```python
from build123d import *

# Parameters (mm, degrees)
SKETCH1_W             = 80
SKETCH1_H             = 105
BOSS_EXTRUDE1_DEPTH   = 3
SKETCH2_R             = 2.6
SKETCH2_R_2           = 15.25
CUT_EXTRUDE1_DEPTH    = 10
M5_TAPPED_HOLE1_D     = 4.2
M5_TAPPED_HOLE1_DEPTH = 12.4
M5_TAPPED_HOLE1_TIP   = 1.2618073
CHAMFER1_SIZE         = 2
SKETCH6_R             = 2.75
CUT_EXTRUDE3_DEPTH    = 133.037873355


with BuildPart() as part:
    # Sketch1 → Boss-Extrude1 (new body)
    with BuildSketch(Plane.XY):
        with Locations((40, 52.5)):
            Rectangle(SKETCH1_W, SKETCH1_H)
    extrude(amount=BOSS_EXTRUDE1_DEPTH)

    # Sketch2 → Cut-Extrude1 (cut)
    with BuildSketch(Plane.XY.offset(3)):
        with Locations((7.5, 97.5)):
            Circle(SKETCH2_R)
        with Locations((72.5, 97.5)):
            Circle(SKETCH2_R)
        with Locations((7.5, 7.5)):
            Circle(SKETCH2_R)
        with Locations((72.5, 7.5)):
            Circle(SKETCH2_R)
        with Locations((40, 65)):
            Circle(SKETCH2_R_2)
    extrude(amount=-CUT_EXTRUDE1_DEPTH, mode=Mode.SUBTRACT)

    # M5 Tapped Hole1
    with Locations(Plane.XY.offset(3)):
        with Locations((11.008621971, 78.991378029), (68.991378029, 78.991378029), (11.008621971, 21.008621971), (68.991378029, 21.008621971)):
            Hole(M5_TAPPED_HOLE1_D / 2, depth=M5_TAPPED_HOLE1_DEPTH)
            with Locations((0, 0, -(M5_TAPPED_HOLE1_DEPTH + M5_TAPPED_HOLE1_TIP / 2))):  # 118° drill point
                Cone(0, M5_TAPPED_HOLE1_D / 2, M5_TAPPED_HOLE1_TIP, mode=Mode.SUBTRACT)

    # Chamfer1
    chamfer1_edges = [part.edges().sort_by_distance(p)[0] for p in [
        (0, 105, 1.5),
        (80, 105, 1.5),
        (80, 0, 1.5),
        (0, 0, 1.5),
    ]]
    chamfer(chamfer1_edges, length=CHAMFER1_SIZE)

    # Sketch6 → Cut-Extrude3 (cut, through all)
    with BuildSketch(Plane(origin=(0, 0, 0), x_dir=(-1, 0, 0), z_dir=(0, 0, -1))):
        with Locations((-68.991378029, 78.991378029)):
            Circle(SKETCH6_R)
        with Locations((-11.008621971, 78.991378029)):
            Circle(SKETCH6_R)
        with Locations((-68.991378029, 21.008621971)):
            Circle(SKETCH6_R)
        with Locations((-11.008621971, 21.008621971)):
            Circle(SKETCH6_R)
    extrude(amount=-CUT_EXTRUDE3_DEPTH, mode=Mode.SUBTRACT)


solid = part.part
```
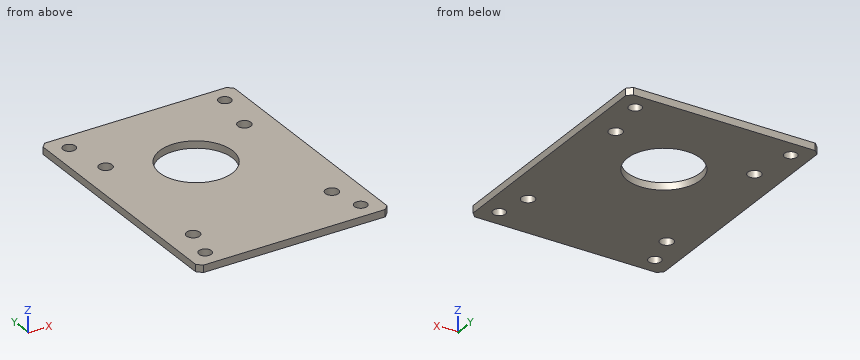
Design review of the part built by this model. Coordinates are the model's own, in mm. Round coordinates to 2 decimals unless told otherwise and drop trailing zeros. Write each loop counter-clockwise with the first axis right and the second up, starting at its lowest first coordinate (ties: lowest second). Pieces come first, ordered by that corner, then holes. Notation, with made-up numbers: (-15.75, -20) -> (21.25, -20) arc R17 cw to (21.25, 6) -> close; hole circle Ø1 at (-3.5, -5). An arc over 180 degrees is marked (long way). Answer in a Markdown table with one row per item.
Q1. To check wall thickness, follow L1, parallel to Y at x = 72.5, z = 1.3; L2, parallel to X at y = 19, z = 2.9; L3, parallel to Y at x = 74.5, z = 1.9. State the ranges of each line that lie inside material, in increasing order. Write a range as [from, to].
The answers:
| item | result |
|---|---|
| L1 | [0, 4.9], [10.1, 94.9], [100.1, 105] |
| L2 | [0, 9.13], [12.89, 67.11], [70.87, 80] |
| L3 | [0, 5.84], [9.16, 95.84], [99.16, 105] |
Q2. Take a section at C-C, the plane y = 65. State the section outline as (x, z) points.
The answers:
| item | result |
|---|---|
| outline | (0, 0) -> (24.75, 0) -> (24.75, 3) -> (0, 3) -> close; (55.25, 0) -> (80, 0) -> (80, 3) -> (55.25, 3) -> close |
Q3. Take a section at A-A, the plane y = 97.5. State the section outline as (x, z) points, then the cut area to 3 significant figures.
The answers:
| item | result |
|---|---|
| outline | (0, 0) -> (4.9, 0) -> (4.9, 3) -> (0, 3) -> close; (10.1, 0) -> (69.9, 0) -> (69.9, 3) -> (10.1, 3) -> close; (75.1, 0) -> (80, 0) -> (80, 3) -> (75.1, 3) -> close |
| area | 209 mm² |
Q4. Take a section at D-D, the plane z = 1.65. Count the separate pieces of the cut face and the enclosed holes in it, then the cut area to 3 significant figures.
The answers:
| item | result |
|---|---|
| separate pieces | 1 |
| enclosed holes | 9 |
| area | 7,480 mm² |
Q5. Take a section at B-B, the plane x = 40. State the section outline as (y, z) points.
The answers:
| item | result |
|---|---|
| outline | (0, 0) -> (49.75, 0) -> (49.75, 3) -> (0, 3) -> close; (80.25, 0) -> (105, 0) -> (105, 3) -> (80.25, 3) -> close |
